Check sheet for the modelled part. Datum: model origin and axes. Units: mm. A direction names the side the tool comes from. Give positions to 0.01 mm unless a question says otherwise; leave off trailing zeros. Loops run counter-clockwise (first coordinate to the right, second up) from the corner with the lowest first, then second, coordinate; pieces in that order, holes last. Notation, with made-up numbers: (58, 36.25) - (100, 36.25) arc R17 cw to (100, 48.25) - close; hole circle Ø8 at (6.5, 21.25). An arc over 180 degrees is marked (long way). Use one line per item in the form item = value.
from build123d import *

# Parameters (mm, degrees)
CUT_EXTRUDE1_DEPTH = 2
FILLET1_R          = 0.5
CHAMFER1_SIZE      = 0.1
CHAMFER1_SIZE2     = 0.567128182
CHAMFER2_SIZE      = 0.5


with BuildPart() as part:
    # Sketch1 → Revolve1 (revolve)
    with BuildSketch(Plane.XY, mode=Mode.PRIVATE) as revolve1_sk:
        Polygon((0, 0), (0, 3.5), (4, 3.5), (4, 2), (16, 2), (16, 0), align=None)
    revolve(revolve1_sk.sketch.rotate(Axis((-4.709244637, 0, 0), (1, 0, 0)), 90), axis=Axis((-4.709244637, 0, 0), (1, 0, 0)))

    # Sketch4 → Cut-Extrude1 (cut)
    with BuildSketch(Plane.ZY):
        Polygon((-1.732050808, 0), (-0.866025404, -1.5), (0.866025404, -1.5), (1.732050808, 0), (0.866025404, 1.5), (-0.866025404, 1.5), align=None)
    extrude(amount=-CUT_EXTRUDE1_DEPTH, mode=Mode.SUBTRACT)

    # Fillet1
    fillet1_edges = [part.edges().sort_by_distance(p)[0] for p in [
        (4, 0, -3.5),
        (0, 0, -3.5),
    ]]
    fillet(fillet1_edges, radius=FILLET1_R)

    # Chamfer1
    chamfer1_edges = [part.edges().sort_by_distance(p)[0] for p in [
        (0, 0.75, -1.299038106),
        (0, -0.75, -1.299038106),
        (0, -1.5, 0),
        (0, -0.75, 1.299038106),
        (0, 0.75, 1.299038106),
        (0, 1.5, 0),
    ]]
    chamfer1_side = [part.faces().sort_by_distance(p)[0] for p in [
        (0, 0, -2.915147186),
    ]]
    chamfer(chamfer1_edges, length=CHAMFER1_SIZE, length2=CHAMFER1_SIZE2, reference=chamfer1_side[0])

    # Chamfer2
    chamfer2_edges = [part.edges().sort_by_distance(p)[0] for p in [
        (16, 0, -2),
    ]]
    chamfer(chamfer2_edges, length=CHAMFER2_SIZE)


solid = part.part
Item 1: Thickness scan on L1, parallel to X at y = -0.75, z = 2.75; L2, parallel to X at y = 0.5, z = 1; L3, parallel to Z at x = 7.5, y = -1. Record the ranges inside material, lowest first.
Answer block:
L1 = 0 to 4
L2 = 2 to 16
L3 = -1.73 to 1.73
Item 2: Section check B-B on x = 8.5. Record the boundary of the cut face in (y, z), then the cut area to 3 significant figures.
Answer block:
outline = circle Ø4 at (0, 0)
area = 12.6 mm2
Item 3: Mould release check, pull along Y, two halves, no side actions. Record for faces 4 (the face through (10, 2, 0)), 5 (the face through (1.274, -0.76, 1.293)), 6 (the face through (0, 1.3, -1.3)): released by +Y, released by -Y, zero draft, split by the parting line, or undercut.
Answer block:
face_4 = split by the parting line
face_5 = undercut
face_6 = zero draft
Item 4: Access from +Z, -Z, +X, -X, +Y, -Y to the whole of each face (thin tool, end or side, straight path). Record for faces 1 (the face through (2.021, 3.105, 1.615)), 2 (the face through (0.29, -0.76, -1.35)), 3 (the face through (4, 2, 1)).
Answer block:
face_1 = +X, -X
face_2 = -X
face_3 = +X
Item 5: Section check A-A on z = 0. Record the boundary of the cut face in (x, y).
Answer block:
outline = (0, -3) arc R0.5 ccw to (0.5, -3.5) - (3.5, -3.5) arc R0.5 ccw to (4, -3) - (4, -2) - (15.5, -2) - (16, -1.5) - (16, 1.5) - (15.5, 2) - (4, 2) - (4, 3) arc R0.5 ccw to (3.5, 3.5) - (0.5, 3.5) arc R0.5 ccw to (0, 3) - (0, 1.6) - (0.57, 1.5) - (2, 1.5) - (2, -1.5) - (0.57, -1.5) - (0, -1.6) - close
Item 6: Gauge pin test, flat ends, axial feed: P1, Ø1.5, axis at y = 0.5, z = 0, coming from the -X side; P2, Ø2, axis at x = 4.5, z = -2.5, coming from the -Y side; P3, Ø4, axis at x = 6.5, z = 2, coming from the -Y side. Record the tip position at first contact, or that the pin passes through.
Answer block:
P1 = 2
P2 = -2.9
P3 = -2
